```python
from build123d import *

# Parameters (mm, degrees)
EXTRUDE_1_DEPTH     = 210
CHAMFER_1_SIZE      = 60
CHAMFER_2_SIZE      = 20
CUT_EXTRUDE_1_DEPTH = 417
SKETCH_4_W          = 80
SKETCH_4_H          = 90.775966299
CUT_EXTRUDE_2_DEPTH = 269


with BuildPart() as part:
    # 草图1 → 凸台-拉伸1 (new body)
    with BuildSketch(Plane.XY):
        with BuildLine():
            Line((0, 0), (0, -115))
            ThreePointArc((0, -115), (2.928932188, -122.071067812), (10, -125))
            Line((10, -125), (180, -125))
            ThreePointArc((180, -125), (187.071067812, -122.071067812), (190, -115))
            Line((190, -115), (190, 0))
            Line((190, 0), (184, 0))
            Line((184, 0), (184, -115))
            ThreePointArc((184, -115), (182.828427125, -117.828427125), (180, -119))
            Line((180, -119), (10, -119))
            ThreePointArc((10, -119), (7.171572875, -117.828427125), (6, -115))
            Line((6, -115), (6, 0))
            Line((6, 0), (0, 0))
        make_face()
    extrude(amount=EXTRUDE_1_DEPTH)

    # 倒角1
    chamfer_1_edges = [part.edges().sort_by_distance(p)[0] for p in [
        (187, 0, 210),
        (3, 0, 210),
    ]]
    chamfer(chamfer_1_edges, length=CHAMFER_1_SIZE)

    # 倒角2
    chamfer_2_edges = [part.edges().sort_by_distance(p)[0] for p in [
        (187, 0, 0),
        (3, 0, 0),
    ]]
    chamfer(chamfer_2_edges, length=CHAMFER_2_SIZE)

    # 草图3 → 切除-拉伸1 (cut)
    with BuildSketch(Plane.XZ.offset(125)):
        with BuildLine():
            Line((34.5, 180.5), (34.5, 139.5))
            ThreePointArc((34.5, 139.5), (30, 135), (25.5, 139.5))
            Line((25.5, 139.5), (25.5, 180.5))
            ThreePointArc((25.5, 180.5), (30, 185), (34.5, 180.5))
        make_face()
        with BuildLine():
            Line((164.5, 180.5), (164.5, 139.5))
            ThreePointArc((164.5, 139.5), (160, 135), (155.5, 139.5))
            Line((155.5, 139.5), (155.5, 180.5))
            ThreePointArc((155.5, 180.5), (160, 185), (164.5, 180.5))
        make_face()
        with BuildLine():
            Line((34.5, 70.5), (34.5, 29.5))
            ThreePointArc((34.5, 29.5), (30, 25), (25.5, 29.5))
            Line((25.5, 29.5), (25.5, 70.5))
            ThreePointArc((25.5, 70.5), (30, 75), (34.5, 70.5))
        make_face()
        with BuildLine():
            Line((164.5, 70.5), (164.5, 29.5))
            ThreePointArc((164.5, 29.5), (160, 25), (155.5, 29.5))
            Line((155.5, 29.5), (155.5, 70.5))
            ThreePointArc((155.5, 70.5), (160, 75), (164.5, 70.5))
        make_face()
    extrude(amount=-CUT_EXTRUDE_1_DEPTH, mode=Mode.SUBTRACT)

    # 草图4 → 切除-拉伸2 (cut)
    with BuildSketch(Plane(origin=(190, 0, 0), x_dir=(0, 0, -1), z_dir=(1, 0, 0))):
        with Locations((-70, -9.61201685)):
            Rectangle(SKETCH_4_W, SKETCH_4_H)
    extrude(amount=-CUT_EXTRUDE_2_DEPTH, mode=Mode.SUBTRACT)


solid = part.part
```
Read the model definition and answer for the solid it produces. Units are mm, in the model's axes. A direction names the side the tool comes from. Round coordinates to 2 decimals unless told otherwise and drop trailing zeros. Write each loop counter-clockwise with the first axis right and the second up, starting at its lowest first coordinate (ties: lowest second). Pieces come first, ordered by that corner, then holes. Notation, with made-up numbers: (-5.5, 37.5) -> (24.5, 37.5) arc R21 ccw to (24.5, 42.5) -> close; hole circle Ø9 at (9, 21). An arc over 180 degrees is marked (long way). Answer in a Markdown table with one row per item. Add a question column.
1) Consider line 1 (X direction, y = -95.5, z = 9.5); line 2 (Y direction, x = 140, z = 171). Determine where each line is inside the solid, lowest interval first.
2) Find section D-D, the plane z = 130. Determine the outline of the cut face in (x, y), and give its area (3 significant figures).
3) Find section A-A, the plane y = -90. Determine the outline of the cut face in (x, z), and give its area (3 significant figures).
4) Find section C-C, the plane x = 160. Determine the outline of the cut face in (y, z), and give its area (3 significant figures).
5) Given P1, Ø3, axis at x = 187, y = -38.5, coming from the +Z side; P2, Ø6.5, axis at y = -120.5, z = 53.5, coming from the +X side; P3, Ø4, axis at x = 65.5, z = 75.5, coming from the +Y side; P4, Ø5, axis at x = 31, z = 140.5, coming from the -Y side, each flat-ended and moving along its own axis, determine where each tip first touches the part or whether it passes through.
6) Find section B-B, the plane z = 41.5. Determine the outline of the cut face in (x, y), and give its area (3 significant figures).
7) Which of the six approach directions +Z, -Z, +X, -X, +Y, -Y give full straight-line access (tool end or side, diameter ignored) to faces 1 (the face through (25.5, -122, 50)), 2 (the face through (3, -55, 71)), 3 (the face through (186.99, -122.15, 103.53))?
Findings below:
| question | item | result |
|---|---|---|
| 1 | line 1 | 0 to 6, 184 to 190 |
| 1 | line 2 | -125 to -119 |
| 2 | outline | (0, -115) arc R10 ccw to (10, -125) -> (180, -125) arc R10 ccw to (190, -115) -> (190, 0) -> (184, 0) -> (184, -115) arc R4 cw to (180, -119) -> (10, -119) arc R4 cw to (6, -115) -> (6, 0) -> (0, 0) -> close |
| 2 | area | 2,530 mm² |
| 3 | outline | (0, 0) -> (6, 0) -> (6, 210) -> (0, 210) -> close; (184, 0) -> (190, 0) -> (190, 210) -> (184, 210) -> close |
| 3 | area | 2,520 mm² |
| 4 | outline | (-125, 0) -> (-119, 0) -> (-119, 25) -> (-125, 25) -> close; (-125, 75) -> (-119, 75) -> (-119, 135) -> (-125, 135) -> close; (-125, 185) -> (-119, 185) -> (-119, 210) -> (-125, 210) -> close |
| 4 | area | 660 mm² |
| 5 | P1 | z = 190 |
| 5 | P2 | x = 189.74 |
| 5 | P3 | y = -119 |
| 5 | P4 | through |
| 6 | outline | (0, -115) arc R10 ccw to (10, -125) -> (25.5, -125) -> (25.5, -119) -> (10, -119) arc R4 cw to (6, -115) -> (6, -55) -> (0, -55) -> close; (34.5, -125) -> (155.5, -125) -> (155.5, -119) -> (34.5, -119) -> close; (164.5, -125) -> (180, -125) arc R10 ccw to (190, -115) -> (190, -55) -> (184, -55) -> (184, -115) arc R4 cw to (180, -119) -> (164.5, -119) -> close |
| 6 | area | 1,760 mm² |
| 7 | face 1 | +Y, -Y |
| 7 | face 2 | +X, -X, +Y |
| 7 | face 3 | +Z, -Z, +X, -Y |
